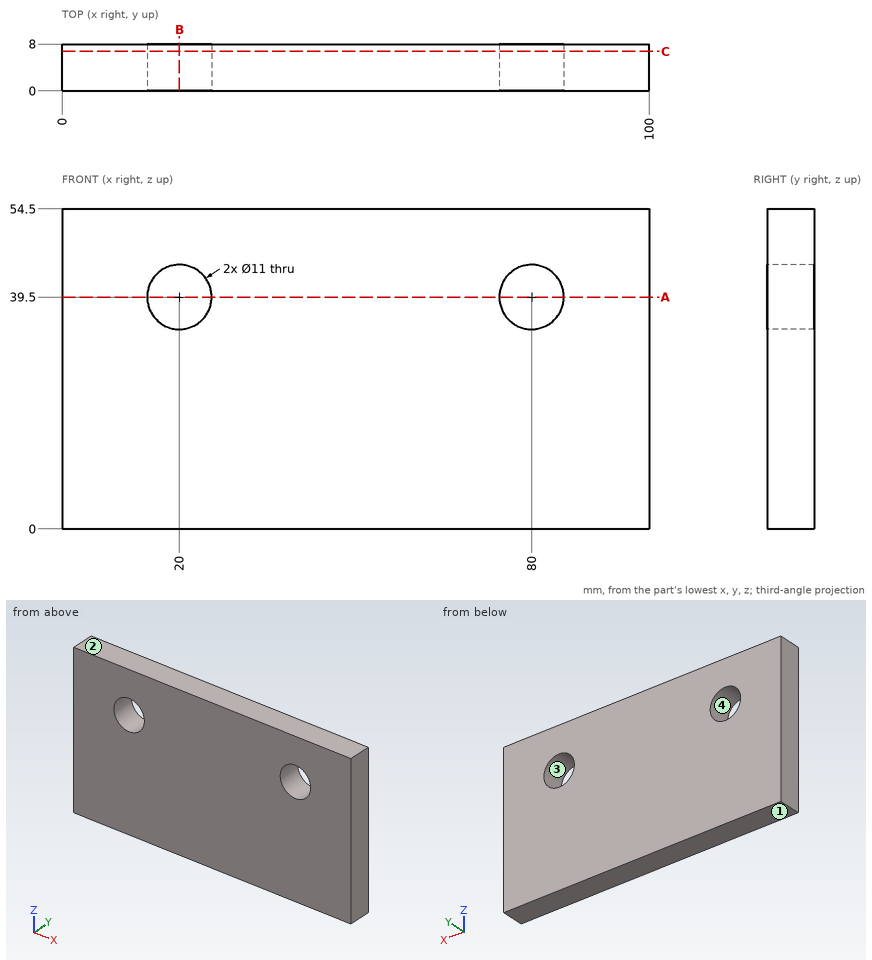
For this review, use the dimensioned drawing (mm, ordinates from the lowest corner) and the shaded views. Round coordinates to 2 decimals unless told otherwise and drop trailing zeros. Write each loop counter-clockwise with the first axis right and the second up, starting at its lowest first coordinate (ties: lowest second). Pieces come first, ordered by that corner, then holes. Notation, with made-up numbers: (-32.5, -39.75) - (-12.5, -39.75) arc R20 cw to (-12.5, -34.75) - close; hole circle Ø7 at (49, -29). An arc over 180 degrees is marked (long way). Answer as a JSON object with one key per item and string values.
1. We need section C-C on y = 6.75. Give the boundary of the cut face in (x, z).
Response values:
{"outline": "(0, 0) - (100, 0) - (100, 54.5) - (0, 54.5) - close; hole circle Ø11 at (20, 39.5); hole circle Ø11 at (80, 39.5)"}
2. To check wall thickness, follow line 1 along X through (y, z) = (6.5, 39); line 2 along Z through (x, y) = (20, 2.25); line 3 along X through (y, z) = (6.25, 43.5). State the ranges of each line that lie inside material, in increasing order.
Response values:
{"line 1": "x = 0 to 14.52, 25.48 to 74.52, 85.48 to 100", "line 2": "z = 0 to 34, 45 to 54.5", "line 3": "x = 0 to 16.23, 23.77 to 76.23, 83.77 to 100"}
3. We need section A-A on z = 39.5. Give the boundary of the cut face in (x, y), then the cut area to 3 significant figures.
Response values:
{"outline": "(0, 0) - (14.5, 0) - (14.5, 8) - (0, 8) - close; (25.5, 0) - (74.5, 0) - (74.5, 8) - (25.5, 8) - close; (85.5, 0) - (100, 0) - (100, 8) - (85.5, 8) - close", "area": "624 mm2"}
4. We need section B-B on x = 20. Give the boundary of the cut face in (y, z), then the cut area to 3 significant figures.
Response values:
{"outline": "(0, 0) - (8, 0) - (8, 34) - (0, 34) - close; (0, 45) - (8, 45) - (8, 54.5) - (0, 54.5) - close", "area": "348 mm2"}
5. Draft analysis for pull direction Z (two halves, no side actions). For the marked faces 1, 2, 3 and 4, state which applies: +Z half, -Z half, draft (parallel to the pull), parting line (faces both ways), or undercut.
Response values:
{"face 1": "-Z half", "face 2": "+Z half", "face 3": "undercut", "face 4": "undercut"}
